```python
from build123d import *

# Parameters (mm, degrees)
BASE_PLATE_DEPTH        = 5
RISER_BLOCK_SKETCH_W    = 40
RISER_BLOCK_SKETCH_H    = 10.827146282
RISER_BLOCK_DEPTH       = 10
UPRIGHT_START           = 35
UPRIGHT_BOSS_35MM_DEPTH = 35
UPRIGHT_START_2         = 45
UPRIGHT_BOSS_45MM_DEPTH = 45
BORE_SKETCH_R           = 5
BORE_CUT_DEPTH          = 22.5
MOUNTING_LUG_DEPTH      = 10
LUG_BOSS_SKETCH_R       = 19
LUG_BOSS_SKETCH_R_2     = 10
LUG_BOSS_DEPTH          = 8


with BuildPart() as part:
    # Base Plate Sketch → Base Plate (new, symmetric)
    with BuildSketch(Plane(origin=(0, 0, 0), x_dir=(1, 0, 0), z_dir=(0, 1, 0))):
        with BuildLine():
            Line((-45, 0), (45, 0))
            Line((45, 0), (45, 28))
            ThreePointArc((45, 28), (48.514718626, 36.485281374), (57, 40))
            Line((57, 40), (60, 40))
            ThreePointArc((60, 40), (68.485281374, 43.514718626), (72, 52))
            Line((72, 52), (72, 75.935046753))
            ThreePointArc((72, 75.935046753), (72.153997607, 76.468225851), (72.568559901, 76.837188339))
            Line((72.568559901, 76.837188339), (75, 78))
            Line((75, 78), (72, 78))
            Line((72, 78), (35, 78))
            Line((35, 78), (35, 61))
            ThreePointArc((35, 61), (34.121320344, 58.878679656), (32, 58))
            Line((32, 58), (-32, 58))
            ThreePointArc((-32, 58), (-34.121320344, 58.878679656), (-35, 61))
            Line((-35, 61), (-35, 78))
            Line((-35, 78), (-72, 78))
            Line((-72, 78), (-75, 78))
            Line((-75, 78), (-72.568559901, 76.837188339))
            ThreePointArc((-72.568559901, 76.837188339), (-72.153997607, 76.468225851), (-72, 75.935046753))
            Line((-72, 75.935046753), (-72, 52))
            ThreePointArc((-72, 52), (-68.485281374, 43.514718626), (-60, 40))
            Line((-60, 40), (-57, 40))
            ThreePointArc((-57, 40), (-48.514718626, 36.485281374), (-45, 28))
            Line((-45, 28), (-45, 0))
        make_face()
    extrude(amount=BASE_PLATE_DEPTH, both=True)

    # Riser Block Sketch → Riser Block (add)
    with BuildSketch(Plane(origin=(0, 5, 0), x_dir=(1, 0, 0), z_dir=(0, 1, 0))):
        with Locations((-55, 83.413573141)):
            Rectangle(RISER_BLOCK_SKETCH_W, RISER_BLOCK_SKETCH_H)
        with Locations((55, 83.413573141)):
            Rectangle(RISER_BLOCK_SKETCH_W, RISER_BLOCK_SKETCH_H)
    extrude(amount=-RISER_BLOCK_DEPTH)

    # Upright Bosses Sketch → Upright Boss 35mm (add)
    with BuildSketch(Plane(origin=(0, 5, 0), x_dir=(1, 0, 0), z_dir=(0, 1, 0)).offset(UPRIGHT_START)):
        with BuildLine():
            Line((0, 53), (0, 58))
            Line((0, 58), (-32, 58))
            ThreePointArc((-32, 58), (-34.121320344, 58.878679656), (-35, 61))
            Line((-35, 61), (-35, 88.827146282))
            Line((-35, 88.827146282), (-75, 88.827146282))
            Line((-75, 88.827146282), (-75, 78.827146282))
            Line((-75, 78.827146282), (-58, 78.827146282))
            ThreePointArc((-58, 78.827146282), (-53.757359313, 77.069786969), (-52, 72.827146282))
            Line((-52, 72.827146282), (-52, 61.686127822))
            ThreePointArc((-52, 61.686127822), (-48.485281374, 53.200846447), (-40, 49.686127822))
            Line((-40, 49.686127822), (-28, 49.686127822))
            ThreePointArc((-28, 49.686127822), (-25.878679656, 48.807448165), (-25, 46.686127822))
            Line((-25, 46.686127822), (-25, 28))
            ThreePointArc((-25, 28), (-17.67766953, 45.67766953), (0, 53))
        make_face()
        with BuildLine():
            Line((75, 78.827146282), (75, 88.827146282))
            Line((75, 88.827146282), (35, 88.827146282))
            Line((35, 88.827146282), (35, 61))
            ThreePointArc((35, 61), (34.121320344, 58.878679656), (32, 58))
            Line((32, 58), (0, 58))
            Line((0, 58), (0, 53))
            ThreePointArc((0, 53), (17.67766953, 45.67766953), (25, 28))
            Line((25, 28), (25, 46.686127822))
            ThreePointArc((25, 46.686127822), (25.878679656, 48.807448165), (28, 49.686127822))
            Line((28, 49.686127822), (40, 49.686127822))
            ThreePointArc((40, 49.686127822), (48.485281374, 53.200846447), (52, 61.686127822))
            Line((52, 61.686127822), (52, 72.827146282))
            ThreePointArc((52, 72.827146282), (53.757359313, 77.069786969), (58, 78.827146282))
            Line((58, 78.827146282), (75, 78.827146282))
        make_face()
    extrude(amount=-UPRIGHT_BOSS_35MM_DEPTH)

    # Sketch5_3 → Upright Boss 45mm (add)
    with BuildSketch(Plane(origin=(0, 5, 0), x_dir=(1, 0, 0), z_dir=(0, 1, 0)).offset(UPRIGHT_START_2)):
        with BuildLine():
            ThreePointArc((25, 28), (17.67766953, 45.67766953), (0, 53))
            Line((0, 53), (0, 43))
            ThreePointArc((0, 43), (10.606601718, 38.606601718), (15, 28))
            ThreePointArc((15, 28), (10.606601718, 17.393398282), (0, 13))
            Line((0, 13), (0, 3))
            ThreePointArc((0, 3), (17.67766953, 10.32233047), (25, 28))
        make_face()
        with BuildLine():
            Line((0, 43), (0, 53))
            ThreePointArc((0, 53), (-17.67766953, 45.67766953), (-25, 28))
            ThreePointArc((-25, 28), (-17.67766953, 10.32233047), (0, 3))
            Line((0, 3), (0, 13))
            ThreePointArc((0, 13), (-15, 28), (0, 43))
        make_face()
        with BuildLine():
            ThreePointArc((25, 28), (17.67766953, 45.67766953), (0, 53))
            Line((0, 53), (0, 43))
            ThreePointArc((0, 43), (10.606601718, 38.606601718), (15, 28))
            ThreePointArc((15, 28), (10.606601718, 17.393398282), (0, 13))
            Line((0, 13), (0, 3))
            ThreePointArc((0, 3), (17.67766953, 10.32233047), (25, 28))
        make_face()
        with BuildLine():
            Line((0, 43), (0, 53))
            ThreePointArc((0, 53), (-17.67766953, 45.67766953), (-25, 28))
            ThreePointArc((-25, 28), (-17.67766953, 10.32233047), (0, 3))
            Line((0, 3), (0, 13))
            ThreePointArc((0, 13), (-15, 28), (0, 43))
        make_face()
    extrude(amount=-UPRIGHT_BOSS_45MM_DEPTH)

    # Bore Sketch → Bore Cut (cut, symmetric)
    with BuildSketch(Plane(origin=(0, 0, -88.827146282), x_dir=(-1, 0, 0), z_dir=(0, 0, -1))):
        with Locations((65, 18)):
            Circle(BORE_SKETCH_R)
        with Locations((-65, 18)):
            Circle(BORE_SKETCH_R)
    extrude(amount=BORE_CUT_DEPTH, both=True, mode=Mode.SUBTRACT)

    # Mounting Lug Sketch → Mounting Lug (add)
    with BuildSketch(Plane.ZY.offset(45)):
        with BuildLine():
            Line((-44.413573141, -5), (-88.827146282, -5))
            Line((-88.827146282, -5), (-63.413573141, -61))
            ThreePointArc((-63.413573141, -61), (-57.848601984, -47.564971157), (-44.413573141, -42))
            Line((-44.413573141, -42), (-44.413573141, -5))
        make_face()
        with BuildLine():
            Line((-28, -5), (-44.413573141, -5))
            Line((-44.413573141, -5), (-44.413573141, -42))
            ThreePointArc((-44.413573141, -42), (-30.978544299, -47.564971157), (-25.413573141, -61))
            Line((-25.413573141, -61), (-16.270280631, -26.90885398))
            ThreePointArc((-16.270280631, -26.90885398), (-11.388179119, -13.538606689), (0, -5))
            Line((0, -5), (-28, -5))
        make_face()
    mounting_lug = extrude(amount=-MOUNTING_LUG_DEPTH)

    # Lug Boss Sketch → Lug Boss (add, symmetric)
    with BuildSketch(Plane.ZY.offset(40)):
        with Locations((-44.413573141, -61)):
            Circle(LUG_BOSS_SKETCH_R)
        with Locations((-44.413573141, -61)):
            Circle(LUG_BOSS_SKETCH_R_2, mode=Mode.SUBTRACT)
    lug_boss = extrude(amount=LUG_BOSS_DEPTH, both=True)

    # Lug Mirror: Mounting Lug, Lug Boss across plane
    add(mounting_lug.mirror(Plane(origin=(0, 0, 0), x_dir=(0, 0, 1), z_dir=(1, 0, 0))))
    add(lug_boss.mirror(Plane(origin=(0, 0, 0), x_dir=(0, 0, 1), z_dir=(1, 0, 0))))


solid = part.part
```
Here's how the part is built. I have some questions about the finished solid (model axes, mm). A direction names the side the tool comes from. Round coordinates to 2 decimals unless told otherwise and drop trailing zeros. Write each loop counter-clockwise with the first axis right and the second up, starting at its lowest first coordinate (ties: lowest second). Pieces come first, ordered by that corner, then holes. Notation, with made-up numbers: M -33.5,32.5 L -16.5,32.5 A31 cw -16.5,67.5 Z; hole C -4,34.5 d1. An arc over 180 degrees is marked long. Answer as CSV lines item,"result". Start each with the question number.
1. I need wall thicknesses on probe 1 along X at (y, z) = (-9, -12); probe 2 along X at (y, z) = (35, -67); probe 3 along Y at (x, z) = (44, -43.5). Which ranges of each line are inside material? Lowest first, please.
2. On a 3-axis mill with a long thin cutter (end or side, diameter ignored), from which of +Z, -Z, +X, -X, +Y, -Y can I reach the whole of each face in a straight line? I mean faces 4 (the flat face through (32, -69, -36)), 5 (the flat face through (0, 18, -58)), 6 (the flat face through (72, 0, -64)). Say none if no direction works.
3. Suppose I cut it at D-D on x = 20. Write out the boundary of the cut face in (y, z).
4. Suppose I cut it at A-A on y = -20. Write out the boundary of the cut face in (x, z), then the cut area to 3 significant figures.
5. Suppose I cut it at B-B on x = -65. Write out the boundary of the cut face in (y, z), then the cut area to 3 significant figures.
6. Thinking about a two-plate mould opening in Z: for faces 1 (the cylindrical face through (-39.888, -67.085, -52.349)), 2 (the flat face through (40.1, -32.6, -76.3)), 3 (the flat face through (-25, 23, -37)), which applies, released by +Z, released by -Z, zero draft, split by the parting line, or undercut?
7. I'm going to push flat-ended pins straight in: pin 1 Ø8 at (y, z) = (-1, -60.5) entering from -X; pin 2 Ø9 at (x, y) = (-65, 18) entering from +Z; pin 3 Ø1 at (x, z) = (-41.5, -28) entering from -Y; pin 4 Ø5 at (x, z) = (-24, -43.5) entering from +Y. Where does each tip first touch, or does it pass through?
8. Suppose I cut it at C-C on y = 26. Write out the boundary of the cut face in (x, z).
Check result:
1,probe 1,"x = -45 to -35, 35 to 45"
1,probe 2,"x = -52 to -35, 35 to 52"
1,probe 3,"y = -79.98 to -70.96, -51.04 to 5"
2,face 4,"+Z, -Z, -Y"
2,face 5,"-Z, +Y, -Y"
2,face 6,"+Z, +X, +Y, -Y"
3,outline,"M -5,-58 L 40,-58 L 40,-43 L 50,-43 L 50,-13 L 5,-13 L 5,0 L -5,0 Z"
4,outline,"M -45,-82.02 L -35,-82.02 L -35,-14.85 L -45,-14.85 Z; M 35,-82.02 L 45,-82.02 L 45,-14.85 L 35,-14.85 Z"
4,area,"1,340 mm2"
5,outline,"M -5,-88.83 L 13,-88.83 L 13,-78.83 L 5,-78.83 L 5,-41.09 L -5,-41.09 Z; M 23,-88.83 L 40,-88.83 L 40,-78.83 L 23,-78.83 Z"
5,area,"727 mm2"
6,face 1,"undercut"
6,face 2,"released by -Z"
6,face 3,"zero draft"
7,pin 1,"stops at x = -72"
7,pin 2,"passes through"
7,pin 3,"stops at y = -71.38"
7,pin 4,"stops at y = 40"
8,outline,"M -75,-88.83 L -35,-88.83 L -35,-61 A3 cw -32,-58 L 32,-58 A3 cw 35,-61 L 35,-88.83 L 75,-88.83 L 75,-78.83 L 58,-78.83 A6 cw 52,-72.83 L 52,-61.69 A12 ccw 40,-49.69 L 28,-49.69 A3 cw 25,-46.69 L 25,-28 A25 ccw -25,-28 L -25,-46.69 A3 cw -28,-49.69 L -40,-49.69 A12 ccw -52,-61.69 L -52,-72.83 A6 cw -58,-78.83 L -75,-78.83 Z; hole C 0,-28 d30"
